Source: CAD feature listing. Evaluate the final solid. Frame: model axes, mm. A direction names the side the tool comes from. Round coordinates to 2 decimals unless told otherwise and drop trailing zeros. Loops run counter-clockwise (first coordinate to the right, second up) from the corner with the lowest first, then second, coordinate; pieces in that order, holes last. Notation, with made-up numbers: M -21.5,63 L 24.5,63 A32 cw 24.5,98 Z; hole C -17.75,63 d5. An arc over 180 degrees is marked long. One line per item, written item: value.
from build123d import *

# Parameters (mm, degrees)
HEX_HEAD_DEPTH              = 45
SHANK_SKETCH_50_R           = 25
SHANK_50X490_DEPTH          = 490
SHANK_END_CHAMFER_4X45_SIZE = 4


with BuildPart() as part:
    # Hex Head Sketch AF104 → Hex Head (new body)
    with BuildSketch(Plane(origin=(0, 0, 0), x_dir=(1, 0, 0), z_dir=(0, 1, 0))):
        Polygon((60.044427996, 0), (30.022213998, 52), (-30.022213998, 52), (-60.044427996, 0), (-30.022213998, -52), (30.022213998, -52), align=None)
    extrude(amount=-HEX_HEAD_DEPTH)

    # Head Chamfer Profile → Head Corner Chamfer Cut (revolve, cut)
    with BuildSketch(Plane.XY, mode=Mode.PRIVATE) as head_corner_chamfer_cut_sk:
        Polygon((50.044427996, 0), (60.044427996, 0), (60.044427996, -10), align=None)
    revolve(head_corner_chamfer_cut_sk.sketch.rotate(Axis((0, 0, 0), (0, -1, 0)), 180.000000001), axis=Axis((0, 0, 0), (0, -1, 0)), mode=Mode.SUBTRACT)

    # Shank Sketch Ø50 → Shank Ø50x490 (add)
    with BuildSketch(Plane(origin=(0, 0, 0), x_dir=(1, 0, 0), z_dir=(0, 1, 0))):
        with Locations(Location((0, 0, 0), (0, 0, 270))):
            Circle(SHANK_SKETCH_50_R)
    extrude(amount=-SHANK_50X490_DEPTH)

    # Shank End Chamfer 4x45°
    shank_end_chamfer_4x45_edges = [part.edges().sort_by_distance(p)[0] for p in [
        (0, -490, -25),
    ]]
    chamfer(shank_end_chamfer_4x45_edges, length=SHANK_END_CHAMFER_4X45_SIZE)


solid = part.part
1. Section query A-A (x = 0). Return the cut outline in (y, z), and give its area (3 significant figures).
Report:
outline: M -490,-21 L -486,-25 L -45,-25 L -45,-52 L -1.96,-52 L 0,-50.04 L 0,50.04 L -1.96,52 L -45,52 L -45,25 L -486,25 L -490,21 Z
area: 26,900 mm2
2. Section query B-B (y = -289). Return the cut outline in (x, z), and give its area (3 significant figures).
Report:
outline: C 0,0 d50
area: 1,960 mm2
3. Ray query, line 1 (Y direction, x = -41.5, z = 27); line 2 (X direction, y = -335.5, z = 13.5); line 3 (Z direction, x = 1.5, y = -103). Return the intervals inside material, ascending. Write a range as [from, to].
Report:
line 1: y = [-45, 0]
line 2: x = [-21.04, 21.04]
line 3: z = [-24.95, 24.95]
4. Pin query (flat end, axial travel): pin 1 (1.5 mm diameter, centred on y = -277, z = 12.5, fed in from -X); pin 2 (1.5 mm diameter, centred on x = -10, y = -335, fed in from +Z); pin 3 (2 mm diameter, centred on x = 15.5, y = -369.5, fed in from -Z). Return the tip coordinate at first contact, or that it passes through.
Report:
pin 1: stops at x = -22.07
pin 2: stops at z = 23.23
pin 3: stops at z = -20.37
5. Reachability of faces 1 (the face through (0, -23, 52)), 2 (the face through (7.509, -262.413, 23.846)) from +Z, -Z, +X, -X, +Y, -Y: full face, straight path, thin tool, end or side. Return the list, or none.
Report:
face 1: +Z, +X, -X, +Y, -Y
face 2: -Y
